Here's how the part is built. I have some questions about the finished solid (model axes, mm). A direction names the side the tool comes from. Give positions to 0.01 mm unless a question says otherwise; leave off trailing zeros. Loops run counter-clockwise (first coordinate to the right, second up) from the corner with the lowest first, then second, coordinate; pieces in that order, holes last.
Q1. For faces 1 (the face through (49, 0, 365)), 2 (the face through (51, 5, 365)), which set-ups out of +Z, -Z, +X, -X, +Y, -Y let a thin tool reach every point of the face, with its end or its side?
Q2. We'd pull the mould along X, two halves only. Please class faces 3 (the face through (100, 24, 365)), 4 (the face through (5, 26, 365)), 5 (the face through (95, 27, 365)), 6 (the face through (50, 2, 0)): +X half, -X half, draft (parallel to the pull), parting line (faces both ways), or undercut.
Q3. If we section it at C-C (x = 88.5): Please give me the cut outline in (y, z).
Q4. I need wall thicknesses on line 1 (X direction, y = 29.5, z = 479.5); line 2 (Y direction, x = 18.5, z = 544). Which ranges of each line are inside material? Lowest first, please.
Q5. Will these pins go through, and if not, where does the flat tip stop? P1, Ø4, axis at x = 3, z = 711, coming from the +Y side; P2, Ø10, axis at x = 67.5, z = 528, coming from the -Y side; P3, Ø1.5, axis at x = 97.5, y = 45, coming from the -Z side; P4, Ø2.5, axis at x = 97, y = 46.5, coming from the +Z side.
Q6. If we section it at A-A (y = 25.5): Please give me the cut outline in (x, z), plus the area to 3 significant figures.
Q7. If we section it at B-B (z = 544.5): Please give me the cut outline in (x, y), plus the area to 3 significant figures.
from build123d import *

# Parameters (mm, degrees)
EXTRUDE_1_DEPTH     = 740
SKETCH_2_W          = 100
SKETCH_2_H          = 5
CUT_EXTRUDE_1_DEPTH = 45
SKETCH_3_W          = 100
SKETCH_3_H          = 5
CUT_EXTRUDE_2_DEPTH = 45
CUT_EXTRUDE_3_DEPTH = 25
CUT_EXTRUDE_4_DEPTH = 25
SKETCH_8_W          = 5
SKETCH_8_H          = 5
CUT_EXTRUDE_5_DEPTH = 25
SKETCH_9_W          = 5
SKETCH_9_H          = 5
CUT_EXTRUDE_6_DEPTH = 25
EXTRUDE_2_DEPTH     = 25
SKETCH_11_W         = 5
SKETCH_11_H         = 5
EXTRUDE_3_DEPTH     = 25
EXTRUDE_4_DEPTH     = 25
SKETCH_13_W         = 5
SKETCH_13_H         = 5
EXTRUDE_5_DEPTH     = 25


with BuildPart() as part:
    # 草图1 → 凸台-拉伸1 (new body)
    with BuildSketch(Plane.XY):
        Polygon((0, 0), (100, 0), (100, 48), (95, 48), (95, 5), (5, 5), (5, 48), (0, 48), align=None)
    extrude(amount=EXTRUDE_1_DEPTH)

    # 草图2 → 切除-拉伸1 (cut)
    with BuildSketch(Plane(origin=(0, 0, 0), x_dir=(-1, 0, 0), z_dir=(0, 0, -1))):
        with Locations((-50, 45.5)):
            Rectangle(SKETCH_2_W, SKETCH_2_H)
    extrude(amount=-CUT_EXTRUDE_1_DEPTH, mode=Mode.SUBTRACT)

    # 草图3 → 切除-拉伸2 (cut)
    with BuildSketch(Plane.XY.offset(740)):
        with Locations((50, 45.5)):
            Rectangle(SKETCH_3_W, SKETCH_3_H)
    extrude(amount=-CUT_EXTRUDE_2_DEPTH, mode=Mode.SUBTRACT)

    # 草图6 → 切除-拉伸3 (cut)
    with BuildSketch(Plane(origin=(0, 0, 0), x_dir=(-1, 0, 0), z_dir=(0, 0, -1))):
        Polygon((-95, 43), (-100, 43), (-100, 0), (0, 0), (0, 43), (-5, 43), (-5, 5), (-95, 5), align=None)
    extrude(amount=-CUT_EXTRUDE_3_DEPTH, mode=Mode.SUBTRACT)

    # 草图7 → 切除-拉伸4 (cut)
    with BuildSketch(Plane.XY.offset(740)):
        Polygon((100, 0), (100, 43), (95, 43), (95, 5), (5, 5), (5, 43), (0, 43), (0, 0), align=None)
    extrude(amount=-CUT_EXTRUDE_4_DEPTH, mode=Mode.SUBTRACT)

    # 草图8 → 切除-拉伸5 (cut)
    with BuildSketch(Plane.XY.offset(695)):
        with Locations((97.5, 45.5)):
            Rectangle(SKETCH_8_W, SKETCH_8_H)
        with Locations((2.5, 45.5)):
            Rectangle(SKETCH_8_W, SKETCH_8_H)
    extrude(amount=-CUT_EXTRUDE_5_DEPTH, mode=Mode.SUBTRACT)

    # 草图9 → 切除-拉伸6 (cut)
    with BuildSketch(Plane(origin=(0, 0, 45), x_dir=(-1, 0, 0), z_dir=(0, 0, -1))):
        with Locations((-2.5, 45.5)):
            Rectangle(SKETCH_9_W, SKETCH_9_H)
        with Locations((-97.5, 45.5)):
            Rectangle(SKETCH_9_W, SKETCH_9_H)
    extrude(amount=-CUT_EXTRUDE_6_DEPTH, mode=Mode.SUBTRACT)

    # 草图10 → 凸台-拉伸2 (add)
    with BuildSketch(Plane(origin=(0, 0, 25), x_dir=(-1, 0, 0), z_dir=(0, 0, -1))):
        Polygon((-95, 5), (-95, 43), (-100, 43), (-100, 0), (0, 0), (0, 43), (-5, 43), (-5, 5), align=None)
    extrude(amount=EXTRUDE_2_DEPTH)

    # 草图11 → 凸台-拉伸3 (add)
    with BuildSketch(Plane(origin=(0, 0, 70), x_dir=(-1, 0, 0), z_dir=(0, 0, -1))):
        with Locations((-2.5, 45.5)):
            Rectangle(SKETCH_11_W, SKETCH_11_H)
        with Locations((-97.5, 45.5)):
            Rectangle(SKETCH_11_W, SKETCH_11_H)
    extrude(amount=EXTRUDE_3_DEPTH)

    # 草图12 → 凸台-拉伸4 (add)
    with BuildSketch(Plane.XY.offset(715)):
        Polygon((0, 0), (100, 0), (100, 43), (95, 43), (95, 5), (5, 5), (5, 43), (0, 43), align=None)
    extrude(amount=EXTRUDE_4_DEPTH)

    # 草图13 → 凸台-拉伸5 (add)
    with BuildSketch(Plane.XY.offset(670)):
        with Locations((2.5, 45.5)):
            Rectangle(SKETCH_13_W, SKETCH_13_H)
        with Locations((97.5, 45.5)):
            Rectangle(SKETCH_13_W, SKETCH_13_H)
    extrude(amount=EXTRUDE_5_DEPTH)


solid = part.part
Check sheet entries:
1. face 1: +Z, -Z, +X, -X, -Y
1. face 2: +Z, -Z, +Y
2. face 3: +X half
2. face 4: undercut
2. face 5: undercut
2. face 6: draft
3. outline: (0, 0) - (5, 0) - (5, 740) - (0, 740) - close
4. line 1: x = 0 to 5, 95 to 100
4. line 2: y = 0 to 5
5. P1: stops at y = 43
5. P2: stops at y = 0
5. P3: stops at z = 45
5. P4: stops at z = 695
6. outline: (0, 0) - (5, 0) - (5, 740) - (0, 740) - close; (95, 0) - (100, 0) - (100, 740) - (95, 740) - close
6. area: 7,400 mm2
7. outline: (0, 0) - (100, 0) - (100, 48) - (95, 48) - (95, 5) - (5, 5) - (5, 48) - (0, 48) - close
7. area: 930 mm2
